from build123d import *

# Parameters (mm, degrees)
SKETCH3_R          = 2.75
CUT_EXTRUDE1_DEPTH = 10
SKETCH4_R          = 4
CUT_EXTRUDE2_DEPTH = 10


with BuildPart() as part:
    # Sketch1 → Revolve1 (revolve)
    with BuildSketch(Plane.XY, mode=Mode.PRIVATE) as revolve1_sk:
        with BuildLine():
            Line((0, -20), (0, -18.5))
            Line((0, -18.5), (-2.878679656, -18.5))
            Line((-2.878679656, -18.5), (-8.5, -12.878679656))
            Line((-8.5, -12.878679656), (-8.5, 3.5))
            Line((-8.5, 3.5), (-5.5, 3.5))
            Line((-5.5, 3.5), (-5.5, 5))
            Line((-5.5, 5), (-8.5, 5))
            Line((-8.5, 5), (-8.5, 14.977248766))
            ThreePointArc((-8.5, 14.977248766), (-13.264398706, 14.628596634), (-18, 14))
            ThreePointArc((-18, 14), (-18.707106781, 13.707106781), (-19, 13))
            Line((-19, 13), (-19, 10.5))
            ThreePointArc((-19, 10.5), (-18.853553391, 10.146446609), (-18.5, 10))
            Line((-18.5, 10), (-14, 10))
            ThreePointArc((-14, 10), (-11.171572875, 8.828427125), (-10, 6))
            Line((-10, 6), (-10, -13.5))
            Line((-10, -13.5), (-3.5, -20))
            Line((-3.5, -20), (0, -20))
        make_face()
    revolve(revolve1_sk.sketch.rotate(Axis((0, 14, 0), (0, -1, 0)), 270), axis=Axis((0, 14, 0), (0, -1, 0)))

    # Sketch3 → Cut-Extrude1 (cut)
    with BuildSketch(Plane.XZ.offset(20)):
        with Locations(Location((0, 0, 0), (0, 0, 270))):
            Circle(SKETCH3_R)
    extrude(amount=-CUT_EXTRUDE1_DEPTH, mode=Mode.SUBTRACT)

    # Sketch4 → Cut-Extrude2 (cut)
    with BuildSketch(Plane.XZ.offset(20)):
        with Locations(Location((0, 0, 0), (0, 0, 90))):
            Circle(SKETCH4_R)
    extrude(amount=-CUT_EXTRUDE2_DEPTH, mode=Mode.SUBTRACT)


solid = part.part
For this review, take the finished solid that the model builds, in its own axes (mm). A direction names the side the tool comes from. Give positions to 0.01 mm unless a question says otherwise; leave off trailing zeros. Loops run counter-clockwise (first coordinate to the right, second up) from the corner with the lowest first, then second, coordinate; pieces in that order, holes last. Notation, with made-up numbers: M 65,-35 L 103,-35 A26 cw 103,0 Z; hole C 56,-21.5 d2. An arc over 180 degrees is marked long. Answer as a JSON object with one key per item and string values. Group by question number.
Q1. Add section A-A on y = 9. Give the boundary of the cut face in (x, z).
Q2. Add section B-B on y = -11. Give the boundary of the cut face in (x, z), and give its area (3 significant figures).
Q3. Tool access review of faces 1 (the cylindrical face through (3.905, -18.454, -0.867)), 2 (the flat face through (-14, 10, -3)), 3 (the flat face through (6, 5, 0)), 4 (the flat face through (6, 3.5, 0)): name each direction out of +Z, -Z, +X, -X, +Y, -Y from which nothing blocks a thin tool from reaching the whole face with its end or side.
Q4. Insertion check: P1, Ø3, axis at y = -9.5, z = 5, coming from the +X side; P2, Ø3, axis at y = 7.5, z = -1.5, coming from the +X side; P3, Ø4, axis at x = 12, y = 10.5, coming from the -Z side. Each pin has a flat end and moves straight along its axis. Give the tip position at first contact, or say it passes through.
Q5. For probe 1 along X at (y, z) = (4, 0); probe 2 along Z at (x, y) = (1.5, 12.5); probe 3 along Z at (x, y) = (-5.5, -9), list the stretches that pass through material, from the lowest coordinate up. Write a range as [from, to].
Q6. Mouldability with a two-part tool opening along Y and no side actions: class faces 5 (the conical face through (-1.3, -19.2, 4.1)), 6 (the cylindrical face through (-8.428, 10.058, -1.107)), 7 (the conical face through (2.6, -17.1, -3.4)) as +Y half, -Y half, draft (parallel to the pull), parting line (faces both ways), or undercut.
Checked values:
{
 "1": {"outline": "C 0,0 d22.71; hole C 0,0 d17"},
 "2": {"outline": "C 0,0 d20; hole C 0,0 d17", "area": "87.2 mm²"},
 "3": {"face 1": "+Y, -Y", "face 2": "-Y", "face 3": "+Y", "face 4": "none"},
 "4": {"P1": "x = 9.37", "P2": "x = 11.27", "P3": "z = -16.16"},
 "5": {"probe 1": "[-10, -5.5], [5.5, 10]", "probe 2": "[-18.94, -8.37], [8.37, 18.94]", "probe 3": "[-8.35, -6.48], [6.48, 8.35]"},
 "6": {"face 5": "-Y half", "face 6": "draft", "face 7": "undercut"}
}
